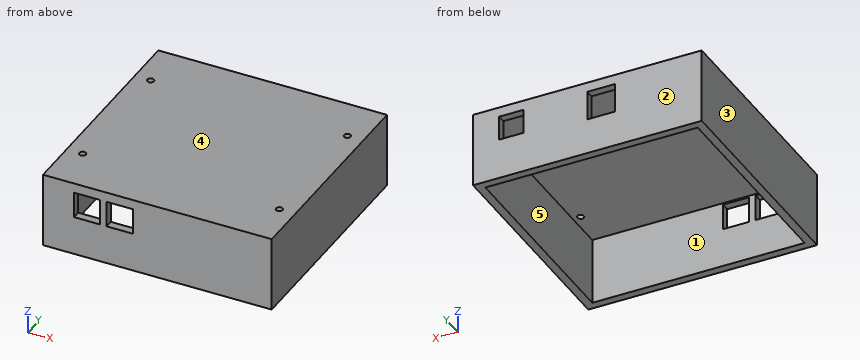
```python
from build123d import *

# Parameters (mm, degrees)
SKETCH1_W           = 140
SKETCH1_H           = 138
BOSS_EXTRUDE1_DEPTH = 46
SHELL1_T            = -5
SKETCH9_W           = 10
SKETCH9_H           = 10
CUT_EXTRUDE2_DEPTH  = 5
SKETCH10_W          = 31
SKETCH10_H          = 22
CUT_EXTRUDE3_DEPTH  = 5
SKETCH11_W          = 17
SKETCH11_H          = 18
CUT_EXTRUDE4_DEPTH  = 5
SKETCH12_W          = 32
SKETCH12_H          = 13
CUT_EXTRUDE5_DEPTH  = 5
SKETCH13_W          = 15
SKETCH13_H          = 15
CUT_EXTRUDE6_DEPTH  = 5
SKETCH19_R          = 2
CUT_EXTRUDE8_DEPTH  = 5
SKETCH21_W          = 16
SKETCH21_H          = 16
CUT_EXTRUDE11_DEPTH = 5
SKETCH23_W          = 16
SKETCH23_H          = 16
CUT_EXTRUDE12_DEPTH = 5
SKETCH24_W          = 10
SKETCH24_H          = 10
SKETCH24_W_2        = 31
SKETCH24_H_2        = 22
SKETCH24_W_3        = 32
SKETCH24_H_3        = 13
BOSS_EXTRUDE2_DEPTH = 5


with BuildPart() as part:
    # Sketch1 → Boss-Extrude1 (new body)
    with BuildSketch(Plane.XY):
        with Locations((22.688228496, 49.11153309)):
            Rectangle(SKETCH1_W, SKETCH1_H)
    extrude(amount=BOSS_EXTRUDE1_DEPTH)

    # Shell1
    shell1_openings = [part.faces().sort_by_distance(p)[0] for p in [
        (22.688228496, 49.11153309, 0),
    ]]
    offset(amount=SHELL1_T, openings=shell1_openings, kind=Kind.INTERSECTION)

    # Sketch9 → Cut-Extrude2 (cut)
    with BuildSketch(Plane(origin=(0, 118.11153309, 0), x_dir=(1, 0, 0), z_dir=(0, 1, 0))):
        with Locations((-34.311771504, -35)):
            Rectangle(SKETCH9_W, SKETCH9_H)
    extrude(amount=-CUT_EXTRUDE2_DEPTH, mode=Mode.SUBTRACT)

    # Sketch10 → Cut-Extrude3 (cut)
    with BuildSketch(Plane(origin=(0, 118.11153309, 0), x_dir=(1, 0, 0), z_dir=(0, 1, 0))):
        with Locations((-11.811771504, -29)):
            Rectangle(SKETCH10_W, SKETCH10_H)
    extrude(amount=-CUT_EXTRUDE3_DEPTH, mode=Mode.SUBTRACT)

    # Sketch11 → Cut-Extrude4 (cut)
    with BuildSketch(Plane(origin=(0, 118.11153309, 0), x_dir=(1, 0, 0), z_dir=(0, 1, 0))):
        with Locations((14.188228496, -31)):
            Rectangle(SKETCH11_W, SKETCH11_H)
    extrude(amount=-CUT_EXTRUDE4_DEPTH, mode=Mode.SUBTRACT)

    # Sketch12 → Cut-Extrude5 (cut)
    with BuildSketch(Plane(origin=(0, 118.11153309, 0), x_dir=(1, 0, 0), z_dir=(0, 1, 0))):
        with Locations((42.688228496, -33.5)):
            Rectangle(SKETCH12_W, SKETCH12_H)
    extrude(amount=-CUT_EXTRUDE5_DEPTH, mode=Mode.SUBTRACT)

    # Sketch13 → Cut-Extrude6 (cut)
    with BuildSketch(Plane(origin=(0, 118.11153309, 0), x_dir=(1, 0, 0), z_dir=(0, 1, 0))):
        with Locations((69.188228496, -32.5)):
            Rectangle(SKETCH13_W, SKETCH13_H)
    extrude(amount=-CUT_EXTRUDE6_DEPTH, mode=Mode.SUBTRACT)

    # Sketch19 → Cut-Extrude8 (cut)
    with BuildSketch(Plane.XY.offset(46)):
        with Locations((-37.511771504, 8.41153309)):
            Circle(SKETCH19_R)
        with Locations((-37.511771504, 89.81153309)):
            Circle(SKETCH19_R)
        with Locations((82.888228496, 8.41153309)):
            Circle(SKETCH19_R)
        with Locations((82.888228496, 89.81153309)):
            Circle(SKETCH19_R)
    extrude(amount=-CUT_EXTRUDE8_DEPTH, mode=Mode.SUBTRACT)

    # Sketch21 → Cut-Extrude11 (cut)
    with BuildSketch(Plane.XZ.offset(19.88846691)):
        with Locations((-20.311771504, 32)):
            Rectangle(SKETCH21_W, SKETCH21_H)
    extrude(amount=-CUT_EXTRUDE11_DEPTH, mode=Mode.SUBTRACT)

    # Sketch23 → Cut-Extrude12 (cut)
    with BuildSketch(Plane.XZ.offset(19.88846691)):
        with Locations((-0.311771504, 32)):
            Rectangle(SKETCH23_W, SKETCH23_H)
    extrude(amount=-CUT_EXTRUDE12_DEPTH, mode=Mode.SUBTRACT)

    # Sketch24 → Boss-Extrude2 (add)
    with BuildSketch(Plane(origin=(0, 118.11153309, 0), x_dir=(1, 0, 0), z_dir=(0, 1, 0))):
        with Locations((-34.311771504, -35)):
            Rectangle(SKETCH24_W, SKETCH24_H)
        with Locations((-11.811771504, -29)):
            Rectangle(SKETCH24_W_2, SKETCH24_H_2)
        with Locations((42.688228496, -33.5)):
            Rectangle(SKETCH24_W_3, SKETCH24_H_3)
    extrude(amount=-BOSS_EXTRUDE2_DEPTH)


solid = part.part
```
Here's how the part is built. I have some questions about the finished solid (model axes, mm). Face numbers are marked on the shaded views. A direction names the side the tool comes from. Give positions to 0.01 mm unless a question says otherwise; leave off trailing zeros. Order: outer loops, then holes, each group sorted by start corner. A loop starts at its lowest first (then second) coordinate and runs counter-clockwise, first axis right, second up. Notation, with made-up numbers: M 26.5,-29.5 L 64.5,-29.5 A27 ccw 64.5,-12.5 Z; hole C -22.5,-13 d3. An arc over 180 degrees is marked long. Use a Markdown table: item, result. Add a question column.
1. Suppose I cut it at D-D (x = 78.5). List the corners of the cut face in (y, z) for me, and give its area (3 significant figures).
2. Suppose I cut it at B-B (z = 31.5). List the corners of the cut face in (x, y) for me, and give its area (3 significant figures).
3. For pin 1 Ø3 at (x, y) = (25.5, 87.5) entering from -Z; pin 2 Ø3 at (x, y) = (-37.51, 8.41) entering from -Z, each with a flat end and sliding along its axis, tell me the tip position at first contact or that it passes through.
4. I need wall thicknesses on probe 1 along X at (y, z) = (88, 38); probe 2 along Y at (x, z) = (53, 30); probe 3 along Y at (x, z) = (10, 39). Which ranges of each line are inside material? Lowest first, please. Write a range as from..to.
5. If we mould it in two halves opening along X, with no side actions, what happens to the marked faces 1, 2 and 3? For each: +X half, -X half, draft (parallel to the pull), parting line (faces both ways), or undercut.
6. On a 3-axis mill with a long thin cutter (end or side, diameter ignored), from which of +Z, -Z, +X, -X, +Y, -Y can I reach the whole of each face in a straight line? I mean the marked faces 4 and 5. Say none if no direction works.
7. Suppose I cut it at C-C (z = 9.5). List the corners of the cut face in (x, y) for me, and give its area (3 significant figures).
8. Suppose I cut it at A-A (x = 19.5). List the corners of the cut face in (y, z) for me, and give its area (3 significant figures).
Results list:
| question | item | result |
|---|---|---|
| 1 | outline | M -19.89,0 L -14.89,0 L -14.89,41 L 113.11,41 L 113.11,0 L 118.11,0 L 118.11,46 L -19.89,46 Z |
| 1 | area | 1,100 mm² |
| 2 | outline | M -47.31,-19.89 L -28.31,-19.89 L -28.31,-14.89 L -42.31,-14.89 L -42.31,113.11 L 5.69,113.11 L 5.69,118.11 L -47.31,118.11 Z; M -12.31,-19.89 L -8.31,-19.89 L -8.31,-14.89 L -12.31,-14.89 Z; M 7.69,-19.89 L 92.69,-19.89 L 92.69,118.11 L 76.69,118.11 L 76.69,113.11 L 87.69,113.11 L 87.69,-14.89 L 7.69,-14.89 Z; M 22.69,113.11 L 61.69,113.11 L 61.69,118.11 L 22.69,118.11 Z |
| 2 | area | 2,360 mm² |
| 3 | pin 1 | stops at z = 41 |
| 3 | pin 2 | passes through |
| 4 | probe 1 | x = -47.31..-42.31, 87.69..92.69 |
| 4 | probe 2 | y = -19.89..-14.89, 113.11..118.11 |
| 4 | probe 3 | y = -19.89..-14.89 |
| 5 | face 1 | undercut |
| 5 | face 2 | draft |
| 5 | face 3 | -X half |
| 6 | face 4 | +Z, +X, -X, +Y, -Y |
| 6 | face 5 | -Z |
| 7 | outline | M -47.31,-19.89 L 92.69,-19.89 L 92.69,118.11 L -47.31,118.11 Z; hole M -42.31,-14.89 L 87.69,-14.89 L 87.69,113.11 L -42.31,113.11 Z |
| 7 | area | 2,680 mm² |
| 8 | outline | M -19.89,0 L -14.89,0 L -14.89,41 L 113.11,41 L 113.11,40 L 118.11,40 L 118.11,46 L -19.89,46 Z; M 113.11,0 L 118.11,0 L 118.11,22 L 113.11,22 Z |
| 8 | area | 1,010 mm² |
